Source: CAD feature listing. Evaluate the final solid. Frame: model axes, mm. A direction names the side the tool comes from. Give positions to 0.01 mm unless a question says otherwise; leave off trailing zeros. Order: outer loops, then holes, each group sorted by start corner. A loop starts at its lowest first (then second) coordinate and runs counter-clockwise, first axis right, second up. Notation, with made-up numbers: M 41.25,-10.5 L 79.25,-10.5 A24 cw 79.25,0.5 Z; hole C -38,27.5 d10. An arc over 180 degrees is marked long. Return JSON: item names as keys, results as strings.
from build123d import *

# Parameters (mm, degrees)
EXTRUDE_1_DEPTH        = 617
HOLE_WIZARD_M4_2_D     = 3.3
HOLE_WIZARD_M4_3_D     = 3.3
HOLE_WIZARD_M4_3_DEPTH = 3
HOLE_WIZARD_M4_1_D     = 4.8
HOLE_WIZARD_M4_4_D     = 3.3
CHAMFER_1_SIZE         = 10


with BuildPart() as part:
    # 草图1 → 凸台-拉伸1 (new, symmetric)
    with BuildSketch(Plane.XY):
        Polygon((0, 0), (60, 0), (60, 60), (57, 60), (57, 3), (0, 3), align=None)
    extrude(amount=EXTRUDE_1_DEPTH, both=True)

    # M4 螺纹孔2 (through all)
    with Locations(Plane(origin=(0, 3, 0), x_dir=(1, 0, 0), z_dir=(0, 1, 0))):
        with Locations((24.75, 499.931449769), (9.75, 484.931449769), (39.75, 484.931449769), (39.75, -484.931449769), (9.75, -484.931449769), (24.75, -499.931449769)):
            Hole(HOLE_WIZARD_M4_2_D / 2)

    # M4 螺纹孔3
    with Locations(Plane(origin=(0, 3, 0), x_dir=(1, 0, 0), z_dir=(0, 1, 0))):
        with Locations((9.75, 484.931449769), (39.75, 484.931449769), (24.75, 469.931449769), (24.75, 499.931449769), (24.75, -499.931449769), (24.75, -469.931449769), (39.75, -484.931449769), (9.75, -484.931449769)):
            Hole(HOLE_WIZARD_M4_3_D / 2, depth=HOLE_WIZARD_M4_3_DEPTH)

    # M4 间隙孔1 (through all)
    with Locations(Plane(origin=(0, 3, 0), x_dir=(1, 0, 0), z_dir=(0, 1, 0))):
        with Locations((42, 0), (42, 200), (42, 400), (42, 600), (42, -600), (42, -400), (42, -200)):
            Hole(HOLE_WIZARD_M4_1_D / 2)

    # M4 螺纹孔4 (through all)
    with Locations(Plane(origin=(0, 3, 0), x_dir=(1, 0, 0), z_dir=(0, 1, 0))):
        with Locations((24.75, 0), (24.75, 120), (24.75, 240), (24.75, 360), (24.75, 480), (24.75, 600), (24.75, -600), (24.75, -480), (24.75, -360), (24.75, -240), (24.75, -120)):
            Hole(HOLE_WIZARD_M4_4_D / 2)

    # 倒角1
    chamfer_1_edges = [part.edges().sort_by_distance(p)[0] for p in [
        (58.5, 60, 617),
        (0, 1.5, 617),
        (58.5, 60, -617),
        (0, 1.5, -617),
    ]]
    chamfer(chamfer_1_edges, length=CHAMFER_1_SIZE)


solid = part.part
1. First-contact query: pin 1 (5 mm diameter, centred on y = 39.5, z = 42.5, fed in from -X); pin 2 (4 mm diameter, centred on x = 24.75, z = -480, fed in from +Y); pin 3 (10 mm diameter, centred on x = 26.5, z = -45, fed in from -Y). Flat tips, straight axial feed; report the tip coordinate or a pass-through.
Evaluation:
{"pin 1": "stops at x = 57", "pin 2": "stops at y = 3", "pin 3": "stops at y = 0"}
2. Section query A-A (z = -99). Return loops of the section in (x, y).
Evaluation:
{"outline": "M 0,0 L 60,0 L 60,60 L 57,60 L 57,3 L 0,3 Z"}
3. Section query B-B (y = 18.5). Return loops of the section in (x, z), then the cut area to 3 significant figures.
Evaluation:
{"outline": "M 57,-617 L 60,-617 L 60,617 L 57,617 Z", "area": "3,700 mm^2"}
4. Ray query, probe 1 along X at (y, z) = (0.7, -600); probe 2 along Z at (x, y) = (39, 1); probe 3 along X at (y, z) = (2.05, -400). Return the intervals inside material, ascending.
Evaluation:
{"probe 1": "x = 0 to 23.1, 26.4 to 39.6, 44.4 to 60", "probe 2": "z = -617 to -486.4, -483.46 to 483.46, 486.4 to 617", "probe 3": "x = 0 to 39.6, 44.4 to 60"}
5. Set-up query: faces 1 (the face through (29, 3, 9)), 2 (the face through (30, 0, 9)). Return all of +Z, -Z, +X, -X, +Y, -Y with unobstructed straight access to the full face (end or side cutting, diameter ignored); none if empty.
Evaluation:
{"face 1": "+Z, -Z, -X, +Y", "face 2": "+Z, -Z, +X, -X, -Y"}
